Build history of the part. All positions in model axes, mm. Give positions to 0.01 mm unless a question says otherwise; leave off trailing zeros. Order: outer loops, then holes, each group sorted by start corner. A loop starts at its lowest first (then second) coordinate and runs counter-clockwise, first axis right, second up. Notation, with made-up numbers: (23, -6.5) - (41, -6.5) arc R34 ccw to (41, 29.5) - close; hole circle Ø4 at (65.5, -32.75). An arc over 180 degrees is marked (long way). Write each question's results on one line, items separated by ' | '. Start each with the question number.
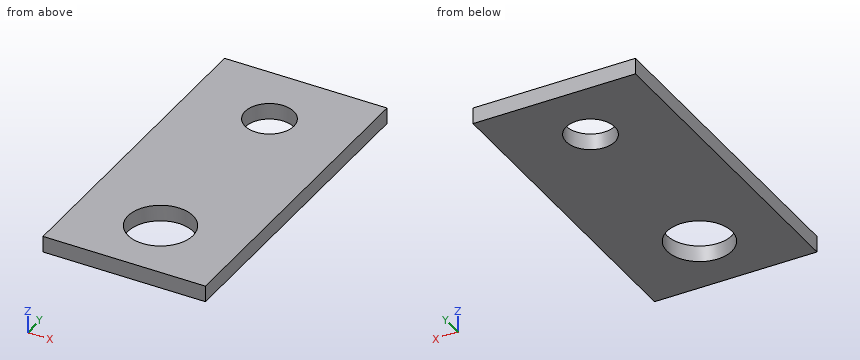
from build123d import *

# Parameters (mm, degrees)
SKETCH1_W           = 50
SKETCH1_H           = 100
BOSS_EXTRUDE1_DEPTH = 5
SKETCH2_R           = 10
SKETCH2_R_2         = 7.5
CUT_EXTRUDE1_DEPTH  = 5


with BuildPart() as part:
    # Sketch1 → Boss-Extrude1 (new body)
    with BuildSketch(Plane.XY):
        Rectangle(SKETCH1_W, SKETCH1_H)
    extrude(amount=BOSS_EXTRUDE1_DEPTH)

    # Sketch2 → Cut-Extrude1 (cut)
    with BuildSketch(Plane.XY.offset(5)):
        with Locations((0, -30)):
            Circle(SKETCH2_R)
        with Locations((0, 30)):
            Circle(SKETCH2_R_2)
    extrude(amount=-CUT_EXTRUDE1_DEPTH, mode=Mode.SUBTRACT)


solid = part.part
Item 1: Cut at B-B, the plane y = -30. List the corners of the cut face in (x, z).
Item 2: Cut at D-D, the plane y = 30. List the corners of the cut face in (x, z).
Item 3: Probe line 1 along Y through (x, z) = (-0.5, 2); line 2 along Y through (x, z) = (5.5, 4.75); line 3 along X through (y, z) = (-34, 2.65). List the from-to ranges inside material, lowest first. Write a range as from..to.
Item 4: Cut at C-C, the plane z = 3.75. List the corners of the cut face in (x, y), then the cut area to 3 significant figures.
Item 5: Cut at A-A, the plane x = 0. List the corners of the cut face in (y, z).
Values found:
1) outline: (-25, 0) - (-10, 0) - (-10, 5) - (-25, 5) - close; (10, 0) - (25, 0) - (25, 5) - (10, 5) - close
2) outline: (-25, 0) - (-7.5, 0) - (-7.5, 5) - (-25, 5) - close; (7.5, 0) - (25, 0) - (25, 5) - (7.5, 5) - close
3) line 1: y = -50..-39.99, -20.01..22.52, 37.48..50 | line 2: y = -50..-38.35, -21.65..24.9, 35.1..50 | line 3: x = -25..-9.17, 9.17..25
4) outline: (-25, -50) - (25, -50) - (25, 50) - (-25, 50) - close; hole circle Ø20 at (0, -30); hole circle Ø15 at (0, 30) | area: 4,510 mm2
5) outline: (-50, 0) - (-40, 0) - (-40, 5) - (-50, 5) - close; (-20, 0) - (22.5, 0) - (22.5, 5) - (-20, 5) - close; (37.5, 0) - (50, 0) - (50, 5) - (37.5, 5) - close
